Job drawing, mm, ordinate dimensions from the low corner. One solid piece. A direction names the side the tool comes from. Give positions to 0.01 mm unless a question says otherwise; leave off trailing zeros. Loops run counter-clockwise (first coordinate to the right, second up) from the corner with the lowest first, then second, coordinate; pieces in that order, holes last. Notation, with made-up numbers: M 45.25,71.25 L 56.25,71.25 A23 cw 56.25,110.25 Z; hole C -19,5.5 d2. An arc over 180 degrees is marked long. Answer in a Markdown table with one row per item.
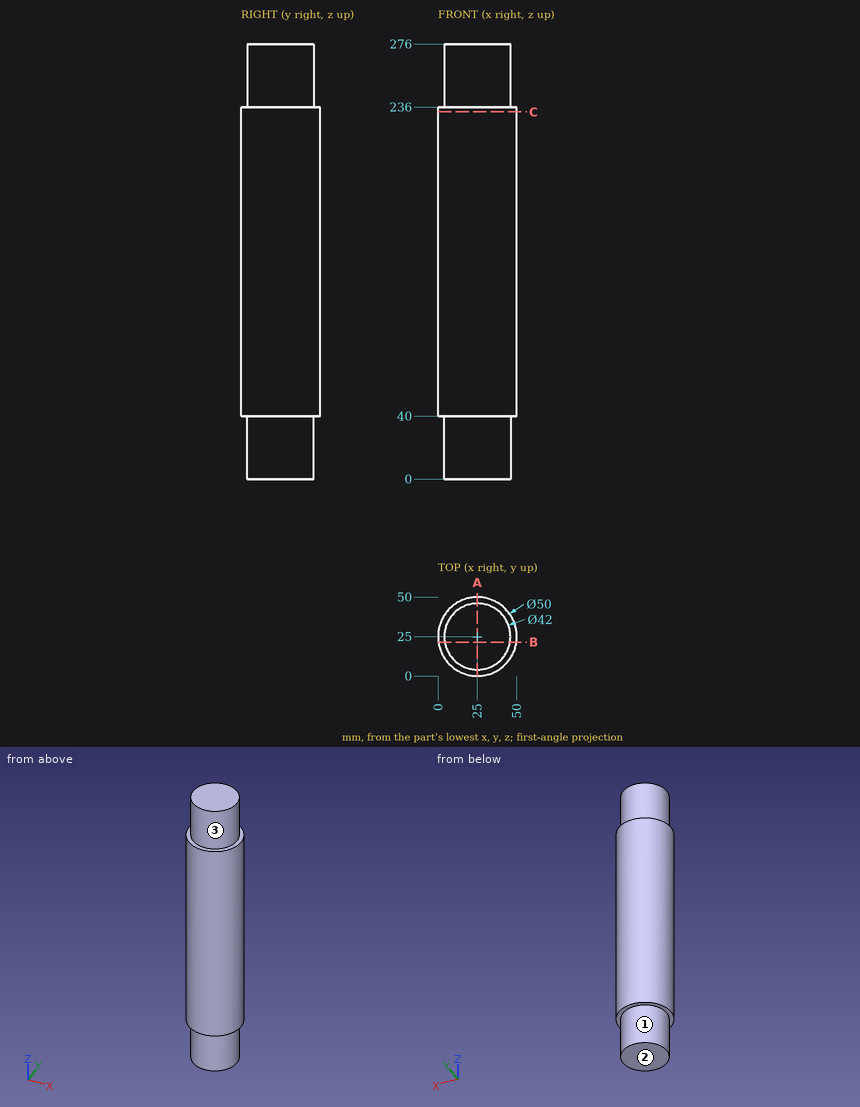
(1) Pin check, flat tips, straight feed: pin 1 Ø5 at (y, z) = (18.5, 132.5) entering from -X; pin 2 Ø12 at (x, y) = (41.5, 44.5) entering from -Z; pin 3 Ø12 at (x, z) = (42.5, 243.5) entering from -Y; pin 4 Ø1.5 at (y, z) = (36.5, 114.5) entering from -X. Stop position of each tip, or through.
Recorded:
| item | result |
|---|---|
| pin 1 | stops at x = 0.32 |
| pin 2 | stops at z = 0 |
| pin 3 | stops at y = 7.43 |
| pin 4 | stops at x = 2.43 |
(2) Saw through at A-A (x = 25). Write the cut outline in (y, z), plus the area to 3 significant figures.
Recorded:
| item | result |
|---|---|
| outline | M 0,40 L 4,40 L 4,0 L 46,0 L 46,40 L 50,40 L 50,236 L 46,236 L 46,276 L 4,276 L 4,236 L 0,236 Z |
| area | 13,200 mm^2 |
(3) Drill centre lines: line 1 along Z through (x, y) = (46, 20.5); line 2 along X through (y, z) = (26, 38); line 3 along X through (y, z) = (47.5, 152). Where is each one in solid material? Low to high.
Recorded:
| item | result |
|---|---|
| line 1 | z = 40 to 236 |
| line 2 | x = 4.02 to 45.98 |
| line 3 | x = 14.1 to 35.9 |
(4) Which spindle directions (+Z, -Z, +X, -X, +Y, -Y) get a long thin tool onto all of the face, cutting with end or side? Do the marked faces 1, 2 and 3. Say none if no direction does.
Recorded:
| item | result |
|---|---|
| face 1 | -Z |
| face 2 | -Z, +X, -X, +Y, -Y |
| face 3 | +Z |
(5) Saw through at B-B (y = 21.5). Write the cut outline in (x, z), plus the area to 3 significant figures.
Recorded:
| item | result |
|---|---|
| outline | M 0.25,40 L 4.29,40 L 4.29,0 L 45.71,0 L 45.71,40 L 49.75,40 L 49.75,236 L 45.71,236 L 45.71,276 L 4.29,276 L 4.29,236 L 0.25,236 Z |
| area | 13,000 mm^2 |
(6) Saw through at C-C (z = 233). Write the cut outline in (x, y), plus the area to 3 significant figures.
Recorded:
| item | result |
|---|---|
| outline | C 25,25 d50 |
| area | 1,960 mm^2 |
